Part model, mm, in its own coordinate system. A direction names the side the tool comes from. Round coordinates to 2 decimals unless told otherwise and drop trailing zeros. Write each loop counter-clockwise with the first axis right and the second up, starting at its lowest first coordinate (ties: lowest second). Pieces come first, ordered by that corner, then holes. Notation, with made-up numbers: (70, 24) -> (112, 24) arc R21 ccw to (112, 62) -> close; hole circle Ø11 at (-23, 10). An arc over 180 degrees is marked (long way). Return JSON: item names as keys, results as strings. Group by question number.
(1) Saw through at A-A (y = 2.05). List the corners of the cut face in (x, z).
(2) Saw through at C-C (y = 0.7). List the corners of the cut face in (x, z).
(3) Drop flat-ended pins along their axis: pin 1 Ø1.6 at (x, z) = (11.35, 3.15) entering from -Y; pin 2 Ø0.8 at (x, z) = (6, 0) entering from -Y; pin 3 Ø4 at (x, z) = (0.5, -1.5) entering from +Y. Give the stop position or say it passes through.
(4) Drill centre lines: L1, parallel to X at y = 2, z = 3.15; L2, parallel to X at y = 0.7, z = 3.15; L3, parallel to X at y = 1.35, z = 0. Where is each one in solid material? Low to high. Write a range as from..to.
(5) Mould opens along Z. For faces 4 (the flat face through (0, 1, 4.15)), 5 (the flat face through (-10, 0, -2)), 6 (the cylindrical face through (-11.66, 1.44, -0.35)) say: +Z half, -Z half, draft (parallel to the pull), parting line (faces both ways), or undercut.
(6) Saw through at B-B (x = 10.1). List the corners of the cut face in (y, z).
(7) Tool access for faces 1 (the flat face through (-4, 0.2, 0)), 2 (the flat face through (12.85, 1, 0)), 3 (the flat face through (4, 2, 0)): list every direction of +Z, -Z, +X, -X, +Y, -Y with a clear straight run to the whole face (end or side of a thin tool).
(8) Saw through at D-D (z = 3.15). State how many separate pieces and enclosed holes the cut face has, plus the area to 3 significant figures.
from build123d import *

# Parameters (mm, degrees)
SKETCH1_W           = 25.7
SKETCH1_H           = 8.3
BOSS_EXTRUDE1_DEPTH = 2.85
SKETCH2_R           = 1.6
SKETCH2_R_2         = 0.6
CUT_EXTRUDE1_DEPTH  = 14.800996341
SKETCH3_W           = 1.7
SKETCH3_H           = 8.3
CUT_EXTRUDE2_DEPTH  = 0.2
SKETCH4_W           = 8
SKETCH4_H           = 8.3
CUT_EXTRUDE3_DEPTH  = 1.35
CHAMFER1_SIZE       = 0.2


with BuildPart() as part:
    # Sketch1 → Boss-Extrude1 (new body)
    with BuildSketch(Plane(origin=(0, 0, 0), x_dir=(1, 0, 0), z_dir=(0, 1, 0))):
        Rectangle(SKETCH1_W, SKETCH1_H)
    extrude(amount=BOSS_EXTRUDE1_DEPTH)

    # Sketch2 → Cut-Extrude1 (cut, through all)
    with BuildSketch(Plane(origin=(0, 2.85, 0), x_dir=(1, 0, 0), z_dir=(0, 1, 0))):
        with Locations(Location((-10.1, 0, 0), (0, 0, 270))):
            Circle(SKETCH2_R)
        with Locations(Location((-11.35, -3.15, 0), (0, 0, 270))):
            Circle(SKETCH2_R_2)
        with Locations(Location((10.1, 0, 0), (0, 0, 90))):
            Circle(SKETCH2_R)
        with Locations(Location((11.35, -3.15, 0), (0, 0, 90))):
            Circle(SKETCH2_R_2)
    extrude(amount=-CUT_EXTRUDE1_DEPTH, mode=Mode.SUBTRACT)

    # Sketch3 → Cut-Extrude2 (cut)
    with BuildSketch(Plane.XZ):
        with Locations((-6.2, 0)):
            Rectangle(SKETCH3_W, SKETCH3_H)
        with Locations((1.2, 0)):
            Rectangle(SKETCH3_W, SKETCH3_H)
        with Locations((-3.8, 0)):
            Rectangle(SKETCH3_W, SKETCH3_H)
        with Locations((-1.2, 0)):
            Rectangle(SKETCH3_W, SKETCH3_H)
        with Locations((3.8, 0)):
            Rectangle(SKETCH3_W, SKETCH3_H)
        with Locations((6.2, 0)):
            Rectangle(SKETCH3_W, SKETCH3_H)
    extrude(amount=-CUT_EXTRUDE2_DEPTH, mode=Mode.SUBTRACT)

    # Sketch4 → Cut-Extrude3 (cut)
    with BuildSketch(Plane(origin=(0, 2.85, 0), x_dir=(1, 0, 0), z_dir=(0, 1, 0))):
        Rectangle(SKETCH4_W, SKETCH4_H)
    extrude(amount=-CUT_EXTRUDE3_DEPTH, mode=Mode.SUBTRACT)

    # Chamfer1
    chamfer1_edges = [part.edges().sort_by_distance(p)[0] for p in [
        (4, 2.85, 0),
        (-4, 2.85, 0),
    ]]
    chamfer(chamfer1_edges, length=CHAMFER1_SIZE)


solid = part.part
Computed values:
{
 "1": {"outline": "(-12.85, -4.15) -> (-4, -4.15) -> (-4, 4.15) -> (-12.85, 4.15) -> close; (4, -4.15) -> (12.85, -4.15) -> (12.85, 4.15) -> (4, 4.15) -> close; hole circle Ø1.2 at (-11.35, 3.15); hole circle Ø3.2 at (-10.1, 0); hole circle Ø3.2 at (10.1, 0); hole circle Ø1.2 at (11.35, 3.15)"},
 "2": {"outline": "(-12.85, -4.15) -> (12.85, -4.15) -> (12.85, 4.15) -> (-12.85, 4.15) -> close; hole circle Ø1.2 at (-11.35, 3.15); hole circle Ø3.2 at (-10.1, 0); hole circle Ø3.2 at (10.1, 0); hole circle Ø1.2 at (11.35, 3.15)"},
 "3": {"pin 1": "y = 0", "pin 2": "y = 0.2", "pin 3": "y = 1.5"},
 "4": {"L1": "-12.85..-11.95, -10.75..-4, 4..10.75, 11.95..12.85", "L2": "-12.85..-11.95, -10.75..10.75, 11.95..12.85", "L3": "-12.85..-11.7, -8.5..8.5, 11.7..12.85"},
 "5": {"face 4": "+Z half", "face 5": "draft", "face 6": "undercut"},
 "6": {"outline": "(0, -4.15) -> (2.85, -4.15) -> (2.85, -1.6) -> (0, -1.6) -> close; (0, 1.6) -> (2.85, 1.6) -> (2.85, 4.15) -> (0, 4.15) -> close"},
 "7": {"face 1": "+Z, -Z, -Y", "face 2": "+Z, -Z, +X, +Y, -Y", "face 3": "+Z, -Z, +Y"},
 "8": {"separate pieces": "3", "enclosed holes": "0", "area": "53.5 mm2"}
}
